```python
from build123d import *

# Parameters (mm, degrees)
BOSS_EXTRUDE1_DEPTH          = 5
M24_TAPPED_HOLE2_D           = 20.4
M24_TAPPED_HOLE2_ON_FACE_2_D = 20.4
HOLE1_D                      = 7
LPATTERN1_COUNT              = 2
LPATTERN1_PITCH              = 80
LPATTERN1_COUNT_DIR2         = 2
LPATTERN1_PITCH_DIR2         = 45


with BuildPart() as part:
    # Sketch1 → Boss-Extrude1 (new body)
    with BuildSketch(Plane(origin=(0, 0, 0), x_dir=(1, 0, 0), z_dir=(0, 1, 0))):
        with BuildLine():
            Line((-35, 32.5), (35, 32.5))
            ThreePointArc((35, 32.5), (45.606601718, 28.106601718), (50, 17.5))
            Line((50, 17.5), (50, -17.5))
            ThreePointArc((50, -17.5), (45.606601718, -28.106601718), (35, -32.5))
            Line((35, -32.5), (-35, -32.5))
            ThreePointArc((-35, -32.5), (-45.606601718, -28.106601718), (-50, -17.5))
            Line((-50, -17.5), (-50, 17.5))
            ThreePointArc((-50, 17.5), (-45.606601718, 28.106601718), (-35, 32.5))
        make_face()
    extrude(amount=BOSS_EXTRUDE1_DEPTH)

    # M24 Tapped Hole2 (through all)
    with Locations(Plane(origin=(0, 0, 0), x_dir=(0, 0, -1), z_dir=(0, -1, 0))):
        with Locations((0, 0)):
            Hole(M24_TAPPED_HOLE2_D / 2)

    # M24 Tapped Hole2 on face 2 (through all)
    with Locations(Plane.ZX.offset(5)):
        with Locations((0, 0)):
            Hole(M24_TAPPED_HOLE2_ON_FACE_2_D / 2)

    # Hole1 (through all)
    with Locations(Plane(origin=(-40, 5, -22.5), x_dir=(0, 0, 1), z_dir=(0, 1, 0))):
        with Locations((0, 0)):
            hole1 = Hole(HOLE1_D / 2)

    # LPattern1: Hole1 2 × 2
    with Locations(*[(i * LPATTERN1_PITCH, 0, j * LPATTERN1_PITCH_DIR2) for i in range(LPATTERN1_COUNT) for j in range(LPATTERN1_COUNT_DIR2) if (i, j) != (0, 0)]):
        add(hole1, mode=Mode.SUBTRACT)


solid = part.part
```
Here's how the part is built. I have some questions about the finished solid (model axes, mm). Coordinates: 2 decimals unless noted, no trailing zeros. Loops run counter-clockwise (first coordinate to the right, second up) from the corner with the lowest first, then second, coordinate; pieces in that order, holes last. Notation, with made-up numbers: M 25,22 L 83,22 A28 cw 83,47 Z; hole C 31,-22.5 d7. An arc over 180 degrees is marked long. One line per item, written item: value.
1. Will these pins go through, and if not, where does the flat tip stop? pin 1 Ø1.5 at (x, z) = (8, 0) entering from +Y; pin 2 Ø1.5 at (y, z) = (2.5, -24.5) entering from +X; pin 3 Ø3 at (y, z) = (2.5, -24) entering from -X.
Geometry says:
pin 1: passes through
pin 2: stops at x = 48.64
pin 3: stops at x = -49.14
2. Imagine slicing it at B-B (x = 0). List the corners of the cut face in (y, z) for me, and give its area (3 significant figures).
Geometry says:
outline: M 0,-32.5 L 5,-32.5 L 5,-10.2 L 0,-10.2 Z; M 0,10.2 L 5,10.2 L 5,32.5 L 0,32.5 Z
area: 223 mm2
3. Imagine slicing it at A-A (z = 0). List the corners of the cut face in (x, y) for me.
Geometry says:
outline: M -50,0 L -10.2,0 L -10.2,5 L -50,5 Z; M 10.2,0 L 50,0 L 50,5 L 10.2,5 Z
4. Thinking about a two-plate mould opening in X: for faces 1 (the flat face through (50, 2, 0)), 2 (the cylindrical face through (-36.53, 2.47, 22.96)), 3 (the cylindrical face through (-45.49, 2.46, 28.22)), which applies, +X half, -X half, draft (parallel to the pull), parting line (faces both ways), or undercut?
Geometry says:
face 1: +X half
face 2: undercut
face 3: -X half
5. Please list where these lines run through material, in increasing order: probe 1 along X at (y, z) = (2.9, 0); probe 2 along X at (y, z) = (2.7, 22); probe 3 along Z at (x, y) = (0, 2.25).
Geometry says:
probe 1: x = -50 to -10.2, 10.2 to 50
probe 2: x = -49.31 to -43.46, -36.54 to 36.54, 43.46 to 49.31
probe 3: z = -32.5 to -10.2, 10.2 to 32.5
6. Imagine slicing it at C-C (y = 3.5). List the corners of the cut face in (x, z) for me, and give its area (3 significant figures).
Geometry says:
outline: M -50,-17.5 A15 ccw -35,-32.5 L 35,-32.5 A15 ccw 50,-17.5 L 50,17.5 A15 ccw 35,32.5 L -35,32.5 A15 ccw -50,17.5 Z; hole C -40,-22.5 d7; hole C -40,22.5 d7; hole C 0,0 d20.4; hole C 40,-22.5 d7; hole C 40,22.5 d7
area: 5,830 mm2
7. Imagine slicing it at D-D (x = -40). List the corners of the cut face in (y, z) for me, and give its area (3 significant figures).
Geometry says:
outline: M 0,-31.64 L 5,-31.64 L 5,-26 L 0,-26 Z; M 0,-19 L 5,-19 L 5,19 L 0,19 Z; M 0,26 L 5,26 L 5,31.64 L 0,31.64 Z
area: 246 mm2
